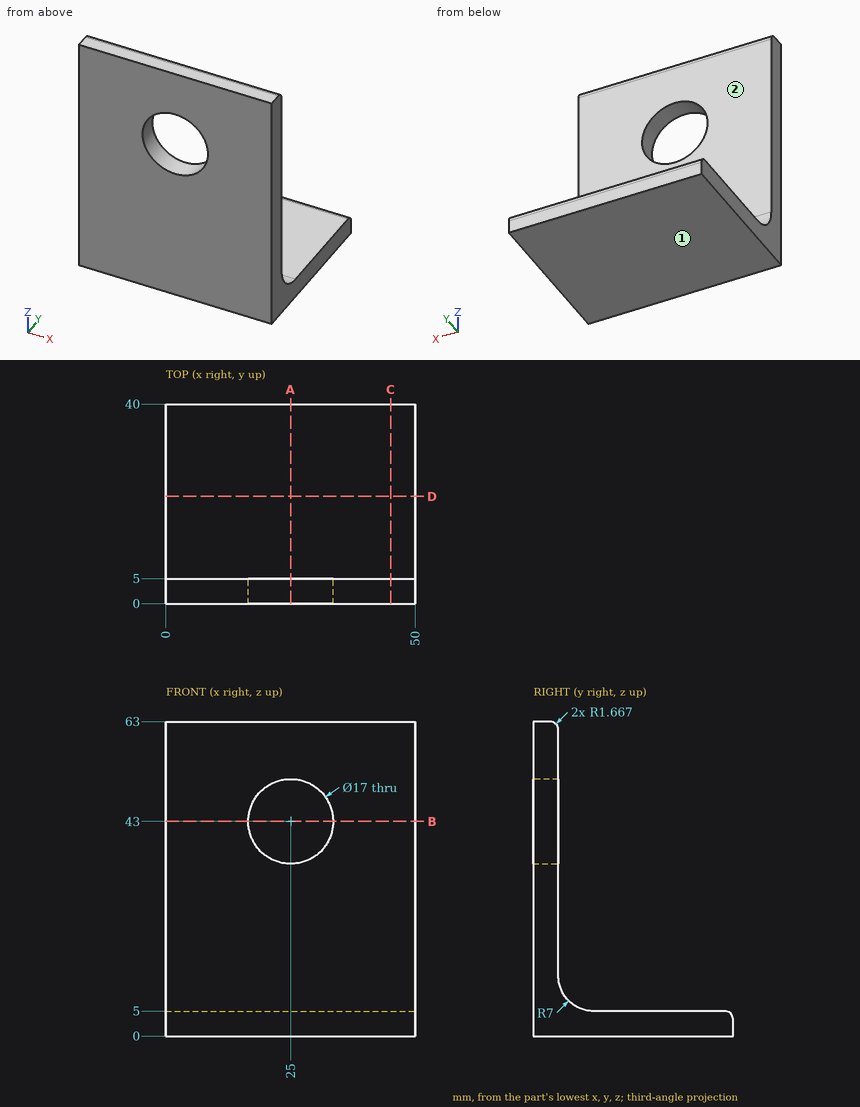
Job drawing, mm, ordinate dimensions from the low corner. One solid piece. A direction names the side the tool comes from. Coordinates: 2 decimals unless noted, no trailing zeros. Order: outer loops, then holes, each group sorted by start corner. A loop starts at its lowest first (then second) coordinate and runs counter-clockwise, first axis right, second up. Notation, with made-up numbers: (56, 21) -> (68, 21) arc R22 ccw to (68, 31) -> close; hole circle Ø9 at (63, -9). An arc over 180 degrees is marked (long way). Put each result on its own line as item: value. Start each with the question number.
(1) Band-saw the part on C-C (x = 45). Give the cut face in (y, z).
(2) Pin check, flat tips, straight feed: pin 1 Ø15 at (x, z) = (23.5, 42) entering from +Y; pin 2 Ø3 at (x, y) = (44, 23.5) entering from +Z. Stop position of each tip, or through.
(3) Band-saw the part on A-A (x = 25). Give the cut face in (y, z), then the cut area to 3 significant figures.
(4) Band-saw the part on B-B (z = 43). Give the cut face in (x, y), then the cut area to 3 significant figures.
(5) Which spindle directions (+Z, -Z, +X, -X, +Y, -Y) get a long thin tool onto all of the face, cutting with end or side? Do the marked faces 1 and 2. Say none if no direction does.
(6) Probe line 1 along X through (y, z) = (1, 43); line 2 along Y through (x, z) = (32.5, 22). List the from-to ranges inside material, lowest first. Write a range as [from, to].
(7) Band-saw the part on D-D (y = 21.5). Give the cut face in (x, z), then the cut area to 3 significant figures.
Determined:
1. outline: (0, 0) -> (40, 0) -> (40, 3.33) arc R1.67 ccw to (38.33, 5) -> (12, 5) arc R7 cw to (5, 12) -> (5, 61.33) arc R1.67 ccw to (3.33, 63) -> (0, 63) -> close
2. pin 1: stops at y = 5
2. pin 2: stops at z = 5
3. outline: (0, 0) -> (40, 0) -> (40, 3.33) arc R1.67 ccw to (38.33, 5) -> (12, 5) arc R7 cw to (5, 12) -> (5, 34.5) -> (0, 34.5) -> close; (0, 51.5) -> (5, 51.5) -> (5, 61.33) arc R1.67 ccw to (3.33, 63) -> (0, 63) -> close
3. area: 414 mm²
4. outline: (0, 0) -> (16.5, 0) -> (16.5, 5) -> (0, 5) -> close; (33.5, 0) -> (50, 0) -> (50, 5) -> (33.5, 5) -> close
4. area: 165 mm²
5. face 1: -Z, +X, -X, +Y, -Y
5. face 2: +Z, +X, -X, +Y
6. line 1: x = [0, 16.5], [33.5, 50]
6. line 2: y = [0, 5]
7. outline: (0, 0) -> (50, 0) -> (50, 5) -> (0, 5) -> close
7. area: 250 mm²
